Could you check a few things on this model? Use its own coordinates, in mm. A direction names the side the tool comes from. Round coordinates to 2 decimals unless told otherwise and drop trailing zeros. Loops run counter-clockwise (first coordinate to the right, second up) from the corner with the lowest first, then second, coordinate; pieces in that order, holes last. Notation, with made-up numbers: (-24, -4) -> (4, -4) arc R26 ccw to (4, 17) -> close; hole circle Ø4 at (-2, 24). An arc over 180 degrees is marked (long way). One line per item, written item: value.
```python
from build123d import *

# Parameters (mm, degrees)
SKETCH1_R           = 21
BOSS_EXTRUDE1_DEPTH = 45
SKETCH8_R           = 19
CUT_EXTRUDE4_DEPTH  = 15
SKETCH2_R           = 20
CUT_EXTRUDE5_DEPTH  = 15
SKETCH6_R           = 5.5
CUT_EXTRUDE6_DEPTH  = 54.916602267
SKETCH10_R          = 21
CUT_EXTRUDE7_DEPTH  = 10
SKETCH13_R          = 21
CUT_EXTRUDE10_DEPTH = 8
CHAMFER4_SIZE       = 3


with BuildPart() as part:
    # Sketch1 → Boss-Extrude1 (new body)
    with BuildSketch(Plane.XY):
        with Locations(Location((0, 0, 0), (0, 0, 180))):
            Circle(SKETCH1_R)
    extrude(amount=BOSS_EXTRUDE1_DEPTH)

    # Sketch8 → Cut-Extrude4 (cut)
    with BuildSketch(Plane.XY.offset(45)):
        Circle(SKETCH8_R)
    extrude(amount=-CUT_EXTRUDE4_DEPTH, mode=Mode.SUBTRACT)

    # Sketch9 → Cut-Revolve2 (revolve, cut)
    with BuildSketch(Plane.XY.offset(30)):
        with BuildLine():
            Line((19, 0), (-19, 0))
            ThreePointArc((-19, 0), (0, 19), (19, 0))
        make_face()
    revolve(axis=Axis((19, 0, 30), (-1, 0, 0)), mode=Mode.SUBTRACT)

    # Sketch2 → Cut-Extrude5 (cut)
    with BuildSketch(Plane.XY.offset(45)):
        Circle(SKETCH2_R)
    extrude(amount=-CUT_EXTRUDE5_DEPTH, mode=Mode.SUBTRACT)

    # Sketch6 → Cut-Extrude6 (cut, through all)
    with BuildSketch(Plane(origin=(0, 0, 0), x_dir=(-1, 0, 0), z_dir=(0, 0, -1))):
        Circle(SKETCH6_R)
    extrude(amount=-CUT_EXTRUDE6_DEPTH, mode=Mode.SUBTRACT)

    # Sketch10 → Cut-Extrude7 (cut)
    with BuildSketch(Plane(origin=(0, 0, 0), x_dir=(-1, 0, 0), z_dir=(0, 0, -1))):
        Circle(SKETCH10_R)
    extrude(amount=-CUT_EXTRUDE7_DEPTH, mode=Mode.SUBTRACT)

    # Sketch13 → Cut-Extrude10 (cut)
    with BuildSketch(Plane(origin=(0, 0, 10), x_dir=(-1, 0, 0), z_dir=(0, 0, -1))):
        Circle(SKETCH13_R)
    extrude(amount=-CUT_EXTRUDE10_DEPTH, mode=Mode.SUBTRACT)

    # Chamfer4
    chamfer4_edges = [part.edges().sort_by_distance(p)[0] for p in [
        (21, 0, 18),
    ]]
    chamfer(chamfer4_edges, length=CHAMFER4_SIZE)


solid = part.part
```
Item 1: Will these pins go through, and if not, where does the flat tip stop? pin 1 Ø4 at (x, y) = (1.5, -15.5) entering from +Z; pin 2 Ø3 at (y, z) = (-15, 31) entering from +X; pin 3 Ø1 at (x, z) = (-5.5, 23) entering from -Y.
Output:
pin 1: stops at z = 22.77
pin 2: stops at x = 16.09
pin 3: stops at y = -20.4
Item 2: If we mould it in two halves opening along Y, with no side actions, what happens to faces 1 (the face through (-19, 8, 45)), 2 (the face through (2.362, 17.991, 18.146)), 3 (the face through (18, -7, 30))? For each: released by +Y, released by -Y, zero draft, split by the parting line, or undercut.
Output:
face 1: zero draft
face 2: split by the parting line
face 3: undercut
Item 3: For faces 4 (the face through (15, 0, 18)), 5 (the face through (-4.336, -19.524, 37.605)), which set-ups out of +Z, -Z, +X, -X, +Y, -Y let a thin tool reach every point of the face, with its end or its side?
Output:
face 4: -Z, +X, -X, +Y, -Y
face 5: +Z
Item 4: I need wall thicknesses on line 1 (Y direction, x = 0, z = 38); line 2 (X direction, y = -7.5, z = 40.25); line 3 (Y direction, x = 14.5, z = 23). Which ranges of each line are inside material? Lowest first, please. Write a range as from..to.
Output:
line 1: y = -21..-20, 20..21
line 2: x = -19.62..-18.54, 18.54..19.62
line 3: y = -15.19..-10.09, 10.09..15.19
Item 5: If we section it at C-C on z = 19.75: List the corners of the cut face in (x, y) for me.
Output:
outline: circle Ø39.5 at (0, 0); hole circle Ø32 at (0, 0)
Item 6: If we section it at A-A on x = 0: List the corners of the cut face in (y, z) for me, plus the area to 3 significant figures.
Output:
outline: (-21, 21) -> (-18, 18) -> (-14.73, 18) arc R19 cw to (-19, 30) -> (-20, 30) -> (-20, 45) -> (-21, 45) -> close; (14.73, 18) -> (18, 18) -> (21, 21) -> (21, 45) -> (20, 45) -> (20, 30) -> (19, 30) arc R19 cw to start
area: 101 mm²
